The model under review builds one solid part; all positions refer to its coordinate system, in mm. A direction names the side the tool comes from. Round coordinates to 2 decimals unless told otherwise and drop trailing zeros. Loops run counter-clockwise (first coordinate to the right, second up) from the corner with the lowest first, then second, coordinate; pieces in that order, holes last. Notation, with made-up numbers: M 46,25 L 95,25 A8 ccw 95,32 Z; hole C 53.5,6.5 d9. An arc over 180 degrees is marked long. One line per question, with ' | ' between items.
from build123d import *

# Parameters (mm, degrees)
SKETCH_1_W                  = 250
SKETCH_1_H                  = 95
EXTRUDE_1_DEPTH             = 10
CUT_EXTRUDE_2_DEPTH         = 135.094183319
PATTERN_LINEAR_1_COUNT      = 2
PATTERN_LINEAR_1_PITCH      = 40
PATTERN_LINEAR_1_COUNT_DIR2 = 2
PATTERN_LINEAR_1_PITCH_DIR2 = 40
PATTERN_LINEAR_2_COUNT      = 2
PATTERN_LINEAR_2_PITCH      = 40
PATTERN_LINEAR_2_COUNT_DIR2 = 2
PATTERN_LINEAR_2_PITCH_DIR2 = 40
CHAMFER_1_SIZE              = 5
HOLE_WIZARD_M10_3_D         = 8.5
HOLE_WIZARD_M10_3_DEPTH     = 24.5
HOLE_WIZARD_M10_3_TIP       = 2.553657631
SKETCH_12_R                 = 13
CUT_EXTRUDE_5_DEPTH         = 135.094183319
HOLE_WIZARD_M6_1_D          = 5
HOLE_WIZARD_M4_1_D          = 3.3
HOLE_WIZARD_M4_1_DEPTH      = 10.1
HOLE_WIZARD_M4_1_TIP        = 0.991420021


with BuildPart() as part:
    # 草图1 → 凸台-拉伸1 (new body)
    with BuildSketch(Plane.XY):
        Rectangle(SKETCH_1_W, SKETCH_1_H)
    extrude(amount=EXTRUDE_1_DEPTH)

    # 草图3 → 切除-拉伸2 (cut, through all)
    with BuildSketch(Plane.XY.offset(10)):
        with BuildLine():
            Line((-59.5, -29.5), (-59.5, -25.5))
            ThreePointArc((-59.5, -25.5), (-55, -21), (-50.5, -25.5))
            Line((-50.5, -25.5), (-50.5, -29.5))
            ThreePointArc((-50.5, -29.5), (-55, -34), (-59.5, -29.5))
        make_face()
    cut_extrude_2 = extrude(amount=-CUT_EXTRUDE_2_DEPTH, mode=Mode.SUBTRACT)

    # 阵列(线性)1: Cut-Extrude 2 2 × 2
    with Locations(*[(i * PATTERN_LINEAR_1_PITCH, j * PATTERN_LINEAR_1_PITCH_DIR2, 0) for i in range(PATTERN_LINEAR_1_COUNT) for j in range(PATTERN_LINEAR_1_COUNT_DIR2) if (i, j) != (0, 0)]):
        add(cut_extrude_2, mode=Mode.SUBTRACT)

    # 阵列(线性)2: Cut-Extrude 2 2 × 2
    with Locations(*[(-i * PATTERN_LINEAR_2_PITCH, j * PATTERN_LINEAR_2_PITCH_DIR2, 0) for i in range(PATTERN_LINEAR_2_COUNT) for j in range(PATTERN_LINEAR_2_COUNT_DIR2) if (i, j) != (0, 0)]):
        add(cut_extrude_2, mode=Mode.SUBTRACT)

    # 倒角1
    chamfer_1_edges = [part.edges().sort_by_distance(p)[0] for p in [
        (125, -47.5, 5),
        (-125, -47.5, 5),
        (-125, 47.5, 5),
        (125, 47.5, 5),
    ]]
    chamfer(chamfer_1_edges, length=CHAMFER_1_SIZE)

    # M10 螺纹孔3
    with Locations(Plane(origin=(42.5, 35, 10), x_dir=(1, 0, 0), z_dir=(0, 0, 1))):
        with Locations((0, 0), (70, 0), (70, -70), (0, -70)):
            Hole(HOLE_WIZARD_M10_3_D / 2, depth=HOLE_WIZARD_M10_3_DEPTH)
            with Locations((0, 0, -(HOLE_WIZARD_M10_3_DEPTH + HOLE_WIZARD_M10_3_TIP / 2))):  # 118° drill point
                Cone(0, HOLE_WIZARD_M10_3_D / 2, HOLE_WIZARD_M10_3_TIP, mode=Mode.SUBTRACT)

    # 草图12 → 切除-拉伸5 (cut, through all)
    with BuildSketch(Plane.XY.offset(10)):
        with Locations((77.5, 0)):
            Circle(SKETCH_12_R)
    extrude(amount=-CUT_EXTRUDE_5_DEPTH, mode=Mode.SUBTRACT)

    # M6 螺纹孔1 (through all)
    with Locations(Plane(origin=(45, -20, 0), x_dir=(-1, 0, 0), z_dir=(0, 0, -1))):
        with Locations((0, 0), (-65, 0), (-65, 40), (0, 40)):
            Hole(HOLE_WIZARD_M6_1_D / 2)

    # M4 螺纹孔1
    with Locations(Plane(origin=(117, -47.5, 5), x_dir=(0, 0, -1), z_dir=(0, -1, 0))):
        with Locations((0, 0), (0, -105), (0, -52.5)):
            Hole(HOLE_WIZARD_M4_1_D / 2, depth=HOLE_WIZARD_M4_1_DEPTH)
            with Locations((0, 0, -(HOLE_WIZARD_M4_1_DEPTH + HOLE_WIZARD_M4_1_TIP / 2))):  # 118° drill point
                Cone(0, HOLE_WIZARD_M4_1_D / 2, HOLE_WIZARD_M4_1_TIP, mode=Mode.SUBTRACT)


solid = part.part
1) Machinability: for faces 4 (the flat face through (-122.5, 45, 4.9)), 5 (the cylindrical face through (-95, -21, 5)), which of the approach directions +Z, -Z, +X, -X, +Y, -Y give a long, thin tool a straight path to every point of the face, cutting with its end or side? Answer none if there is none.
Output values:
face 4: +Z, -Z, -X, +Y | face 5: +Z, -Z
2) Mouldability with a two-part tool opening along X and no side actions: class faces 1 (the flat face through (122.5, 45, 4.9)), 2 (the cylindrical face through (-55, -21, 5)), 3 (the flat face through (-2, 1, 0)) as +X half, -X half, draft (parallel to the pull), parting line (faces both ways), or undercut.
Output values:
face 1: +X half | face 2: undercut | face 3: draft
3) For line 1 (X direction, y = -28, z = 4); line 2 (Z direction, x = 117, y = -44.25); line 3 (X direction, y = 16.5, z = 1.5), list the stretches that pass through material, from the lowest coordinate up.
Output values:
line 1: x = -125 to -99.5, -90.5 to -59.5, -50.5 to -19.5, -10.5 to 125 | line 2: z = 0 to 3.35, 6.65 to 10 | line 3: x = -125 to -99.03, -90.97 to -59.03, -50.97 to -19.03, -10.97 to 125
4) Add section A-A on x = -95. State the section outline as (y, z) points, then the cut area to 3 significant figures.
Output values:
outline: M -47.5,0 L -34,0 L -34,10 L -47.5,10 Z; M -21,0 L 6,0 L 6,10 L -21,10 Z; M 19,0 L 47.5,0 L 47.5,10 L 19,10 Z | area: 690 mm²
5) Add section B-B on x = 77.5. State the section outline as (y, z) points, then the cut area to 3 significant figures.
Output values:
outline: M -47.5,0 L -13,0 L -13,10 L -47.5,10 Z; M 13,0 L 47.5,0 L 47.5,10 L 13,10 Z | area: 690 mm²
6) Insertion check: P1, Ø7, axis at x = 112.5, y = -35, coming from the -Z side. The pin has a flat end and moves straight along its axis. Give the tip position at first contact, or say it passes through.
Output values:
P1: passes through
